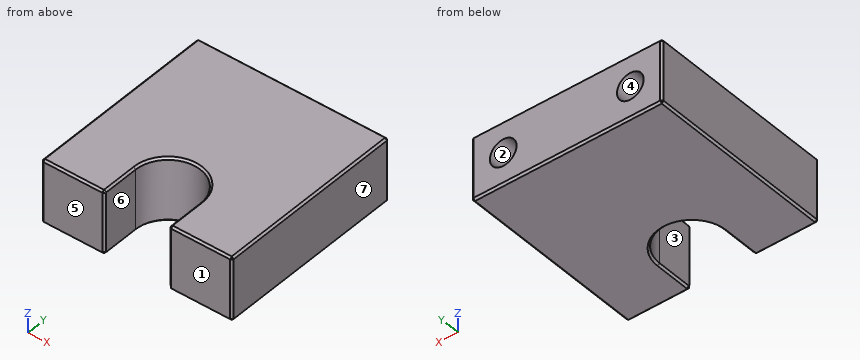
from build123d import *

# Parameters (mm, degrees)
SKETCH_1_W             = 30
SKETCH_1_H             = 30
EXTRUDE_1_DEPTH        = 10
HOLE_WIZARD_M5_1_D     = 4.2
HOLE_WIZARD_M5_1_DEPTH = 16
HOLE_WIZARD_M5_1_TIP   = 1.2618073
CHAMFER_1_SIZE         = 0.3
CUT_EXTRUDE_1_DEPTH    = 24.452078799
CHAMFER_2_SIZE         = 0.3


with BuildPart() as part:
    # 草图1 → 凸台-拉伸1 (new body)
    with BuildSketch(Plane.XY):
        Rectangle(SKETCH_1_W, SKETCH_1_H)
    extrude(amount=EXTRUDE_1_DEPTH)

    # M5 螺纹孔1
    with Locations(Plane(origin=(9.101151333, 15, -0.360612024), x_dir=(-1, 0, 0), z_dir=(0, 1, 0))):
        with Locations((-0.898848667, 5.360612024), (19.101151333, 5.360612024)):
            Hole(HOLE_WIZARD_M5_1_D / 2, depth=HOLE_WIZARD_M5_1_DEPTH)
            with Locations((0, 0, -(HOLE_WIZARD_M5_1_DEPTH + HOLE_WIZARD_M5_1_TIP / 2))):  # 118° drill point
                Cone(0, HOLE_WIZARD_M5_1_D / 2, HOLE_WIZARD_M5_1_TIP, mode=Mode.SUBTRACT)

    # 倒角1
    chamfer_1_edges = [part.edges().sort_by_distance(p)[0] for p in [
        (-15, 0, 10),
        (0, -15, 10),
        (15, 0, 10),
        (0, -15, 0),
        (-15, 0, 0),
        (0, 15, 0),
        (15, 0, 0),
        (0, 15, 10),
        (15, -15, 5),
        (-15, -15, 5),
        (-15, 15, 5),
        (15, 15, 5),
    ]]
    chamfer(chamfer_1_edges, length=CHAMFER_1_SIZE)

    # 草图4 → 切除-拉伸1 (cut, through all)
    with BuildSketch(Plane.XY.offset(10)):
        with BuildLine():
            Line((-5.1, -15), (-5.1, -9))
            ThreePointArc((-5.1, -9), (0, -3.9), (5.1, -9))
            Line((5.1, -9), (5.1, -15))
            ThreePointArc((5.1, -15), (0, -20.1), (-5.1, -15))
        make_face()
    extrude(amount=-CUT_EXTRUDE_1_DEPTH, mode=Mode.SUBTRACT)

    # 倒角2
    chamfer_2_edges = [part.edges().sort_by_distance(p)[0] for p in [
        (5.1, -14.85, 0.15),
        (-5.1, -14.85, 0.15),
        (-5.1, -14.85, 9.85),
        (5.1, -14.85, 9.85),
        (5.1, -15, 5),
        (-5.1, -11.85, 0),
        (-5.1, -15, 5),
        (0, -3.9, 0),
        (5.1, -11.85, 0),
        (5.1, -11.85, 10),
        (0, -3.9, 10),
        (-5.1, -11.85, 10),
    ]]
    chamfer(chamfer_2_edges, length=CHAMFER_2_SIZE)


solid = part.part
The listing builds one solid part. Answer for the finished solid, in the listing's coordinates (mm). Face numbers are marked on the shaded views. A direction names the side the tool comes from. Give positions to 0.01 mm unless a question says otherwise; leave off trailing zeros. Order: outer loops, then holes, each group sorted by start corner. A loop starts at its lowest first (then second) coordinate and runs counter-clockwise, first axis right, second up. Notation, with made-up numbers: (60.5, 71.5) - (105.5, 71.5) arc R18 cw to (105.5, 92.5) - close; hole circle Ø4 at (51.25, 26.25). An arc over 180 degrees is marked (long way). Use one line per item in the form item = value.
1) Find section C-C on z = 8.25. Determine the outline of the cut face in (x, y).
Verdict:
outline = (-15, -14.7) - (-14.7, -15) - (-5.4, -15) - (-5.1, -14.7) - (-5.1, -9) arc R5.1 cw to (5.1, -9) - (5.1, -14.7) - (5.4, -15) - (14.7, -15) - (15, -14.7) - (15, 14.7) - (14.7, 15) - (-14.7, 15) - (-15, 14.7) - close
2) Consider probe 1 along X at (y, z) = (4.5, 5); probe 2 along Z at (x, y) = (10, 3.75); probe 3 along X at (y, z) = (10, 6). Determine where each line is inside the solid, lowest interval first. Write a range as [from, to].
Verdict:
probe_1 = [-15, -12.1], [-7.9, 7.9], [12.1, 15]
probe_2 = [0, 2.9], [7.1, 10]
probe_3 = [-15, -11.85], [-8.15, 8.15], [11.85, 15]
3) Find section B-B on x = 0. Determine the outline of the cut face in (y, z).
Verdict:
outline = (-3.9, 0.3) - (-3.6, 0) - (14.7, 0) - (15, 0.3) - (15, 9.7) - (14.7, 10) - (-3.6, 10) - (-3.9, 9.7) - close
4) For the marked faces 1, 2 and 3, determine the directions among +Z, -Z, +X, -X, +Y, -Y from which every point of the face is accessible in a straight line to the end or side of a thin tool.
Verdict:
face_1 = +Z, -Z, +X, -X, -Y
face_2 = +Y
face_3 = +Z, -Z, -Y
5) Find section A-A on y = 2. Determine the outline of the cut face in (x, z).
Verdict:
outline = (-15, 0.3) - (-14.7, 0) - (14.7, 0) - (15, 0.3) - (15, 9.7) - (14.7, 10) - (-14.7, 10) - (-15, 9.7) - close; hole circle Ø4.2 at (-10, 5); hole circle Ø4.2 at (10, 5)
6) The mould has two halves that part along X. Classify the marked faces 4, 5, 6 and 7: released by +X, released by -X, zero draft, split by the parting line, or undercut.
Verdict:
face_4 = undercut
face_5 = zero draft
face_6 = undercut
face_7 = released by +X
